```python
from build123d import *

# Parameters (mm, degrees)
BOSS_EXTRUDE1_DEPTH          = 1.5
SKETCH2_W                    = 90
SKETCH2_H                    = 1.5
BOSS_EXTRUDE2_DEPTH          = 36
BOSS_EXTRUDE3_DEPTH          = 1.5
F_6_0_6_DIAMETER_HOLE1_D     = 6
F_6_0_6_DIAMETER_HOLE1_DEPTH = 1.5
F_6_0_6_DIAMETER_HOLE2_D     = 6
F_4_0_4_DIAMETER_HOLE1_D     = 4
F_3_0_3_DIAMETER_HOLE1_D     = 3
FILLET1_R                    = 0.7366
FILLET2_R                    = 2.2366


with BuildPart() as part:
    # Sketch1 → Boss-Extrude1 (new body)
    with BuildSketch(Plane(origin=(-29, 0, 0), x_dir=(0, -1, 0), z_dir=(-1, 0, 0))):
        with BuildLine():
            Line((-9.138054181, -90), (1.5, -90))
            Line((1.5, -90), (1.5, 0))
            Line((1.5, 0), (-2.128893479, 0))
            ThreePointArc((-2.128893479, 0), (-9.130094082, -7.130859089), (-2.128893479, -14.261718178))
            Line((-2.128893479, -14.261718178), (-2.128893479, -41.261718178))
            Line((-2.128893479, -41.261718178), (-3.628893479, -41.261718178))
            ThreePointArc((-3.628893479, -41.261718178), (-5.147993713, -42.802982792), (-5.778257675, -44.873231442))
            ThreePointArc((-5.778257675, -44.873231442), (-5.210002115, -47.08061414), (-3.638283373, -48.73141787))
            Line((-3.638283373, -48.73141787), (-2.138054181, -48.73141787))
            Line((-2.138054181, -48.73141787), (-2.138054181, -75.73141787))
            ThreePointArc((-2.138054181, -75.73141787), (-7.103512649, -77.954400774), (-9.138054181, -83))
            Line((-9.138054181, -83), (-9.138054181, -90))
        make_face()
    extrude(amount=-BOSS_EXTRUDE1_DEPTH)

    # Sketch2 → Boss-Extrude2 (add)
    with BuildSketch(Plane(origin=(-27.5, 0, 0), x_dir=(0, 0, -1), z_dir=(1, 0, 0))):
        with Locations((45, -0.75)):
            Rectangle(SKETCH2_W, SKETCH2_H)
    extrude(amount=BOSS_EXTRUDE2_DEPTH)

    # Sketch3 → Boss-Extrude3 (add)
    with BuildSketch(Plane(origin=(8.5, 0, 0), x_dir=(0, 0, -1), z_dir=(1, 0, 0))):
        with BuildLine():
            Line((0, -1.5), (0, 2.128893479))
            ThreePointArc((0, 2.128893479), (7.130859089, 9.130094082), (14.261718178, 2.128893479))
            Line((14.261718178, 2.128893479), (41.261718178, 2.128893479))
            Line((41.261718178, 2.128893479), (41.261718178, 3.628893479))
            ThreePointArc((41.261718178, 3.628893479), (42.802982792, 5.147993713), (44.873231442, 5.778257675))
            ThreePointArc((44.873231442, 5.778257675), (47.08061414, 5.210002115), (48.73141787, 3.638283373))
            Line((48.73141787, 3.638283373), (48.73141787, 2.138054181))
            Line((48.73141787, 2.138054181), (75.73141787, 2.138054181))
            ThreePointArc((75.73141787, 2.138054181), (77.954400774, 7.103512649), (83, 9.138054181))
            Line((83, 9.138054181), (90, 9.138054181))
            Line((90, 9.138054181), (90, -1.5))
            Line((90, -1.5), (0, -1.5))
        make_face()
    extrude(amount=BOSS_EXTRUDE3_DEPTH)

    # Ø6.0 (6) Diameter Hole1
    with Locations(Plane.ZY.offset(-8.5)):
        with Locations((-6.845764439, 4.481725402), (-83, 4.638054181)):
            Hole(F_6_0_6_DIAMETER_HOLE1_D / 2, depth=F_6_0_6_DIAMETER_HOLE1_DEPTH)

    # Ø6.0 (6) Diameter Hole2 (through all)
    with Locations(Plane(origin=(-27.5, 0, 0), x_dir=(0, 0, -1), z_dir=(1, 0, 0))):
        with Locations((83, 4.638054181), (6.845764439, 4.481725402)):
            Hole(F_6_0_6_DIAMETER_HOLE2_D / 2)

    # Ø4.0 (4) Diameter Hole1 (through all)
    with Locations(Plane(origin=(0, 0, 0), x_dir=(1, 0, 0), z_dir=(0, 1, 0))):
        with Locations((-19.5, 76), (0.5, 76)):
            Hole(F_4_0_4_DIAMETER_HOLE1_D / 2)

    # Ø3.0 (3) Diameter Hole1 (through all)
    with Locations(Plane(origin=(0, 0, 0), x_dir=(1, 0, 0), z_dir=(0, 1, 0))):
        with Locations((-9.5, 6), (-9.5, 23)):
            Hole(F_3_0_3_DIAMETER_HOLE1_D / 2)

    # Fillet1
    fillet1_edges = [part.edges().sort_by_distance(p)[0] for p in [
        (-27.5, 0, -45),
        (8.5, 0, -45),
    ]]
    fillet(fillet1_edges, radius=FILLET1_R)

    # Fillet2
    fillet2_edges = [part.edges().sort_by_distance(p)[0] for p in [
        (-29, -1.5, -45),
        (10, -1.5, -45),
    ]]
    fillet(fillet2_edges, radius=FILLET2_R)


solid = part.part
```
Build history of the part. All positions in model axes, mm. A direction names the side the tool comes from. Round coordinates to 2 decimals unless told otherwise and drop trailing zeros. Order: outer loops, then holes, each group sorted by start corner. A loop starts at its lowest first (then second) coordinate and runs counter-clockwise, first axis right, second up. Notation, with made-up numbers: (-30.75, -40) -> (-22.75, -40) arc R18 ccw to (-22.75, -35) -> close; hole circle Ø1 at (49.5, 58). An arc over 180 degrees is marked (long way). Answer in a Markdown table with one row per item.
1) Wall check: L1, parallel to Z at x = -9.5, y = -0.55; L2, parallel to X at y = 4, z = -42; L3, parallel to Y at x = -6, z = -17. Give the ranges that are in metal, low to high.
Values:
| item | result |
|---|---|
| L1 | -90 to -24.5, -21.5 to -7.5, -4.5 to 0 |
| L2 | -29 to -27.5, 8.5 to 10 |
| L3 | -1.5 to 0 |
2) Band-saw the part on D-D on z = -82. Give the cut face in (x, y).
Values:
| item | result |
|---|---|
| outline | (-29, 0.74) arc R2.24 ccw to (-26.76, -1.5) -> (7.76, -1.5) arc R2.24 ccw to (10, 0.74) -> (10, 1.81) -> (8.5, 1.81) -> (8.5, 0.74) arc R0.74 cw to (7.76, 0) -> (-26.76, 0) arc R0.74 cw to (-27.5, 0.74) -> (-27.5, 1.81) -> (-29, 1.81) -> close; (-29, 7.47) -> (-27.5, 7.47) -> (-27.5, 9.07) -> (-29, 9.07) -> close; (8.5, 7.47) -> (10, 7.47) -> (10, 9.07) -> (8.5, 9.07) -> close |
3) Band-saw the part on C-C on z = -32. Give the cut face in (x, y).
Values:
| item | result |
|---|---|
| outline | (-29, 0.74) arc R2.24 ccw to (-26.76, -1.5) -> (7.76, -1.5) arc R2.24 ccw to (10, 0.74) -> (10, 2.13) -> (8.5, 2.13) -> (8.5, 0.74) arc R0.74 cw to (7.76, 0) -> (-26.76, 0) arc R0.74 cw to (-27.5, 0.74) -> (-27.5, 2.13) -> (-29, 2.13) -> close |
4) Pin check, flat tips, straight feed: P1, Ø5.5, axis at y = 4.64, z = -83, coming from the +X side; P2, Ø1.2, axis at x = 9.5, z = -33, coming from the +Y side; P3, Ø10.5, axis at x = -2.5, z = -42.5, coming from the +Y side. Stop position of each tip, or through.
Values:
| item | result |
|---|---|
| P1 | through |
| P2 | y = 2.13 |
| P3 | y = 0 |
5) Mould opens along Y. For faces 4 (the cylindrical face through (-28.26, 9.13, -6.98)), 5 (the flat face through (9, 3, -41.262)), 6 (the cylindrical face through (9.26, 7.01, -8.46)) say: released by +Y, released by -Y, zero draft, split by the parting line, or undercut.
Values:
| item | result |
|---|---|
| face 4 | released by +Y |
| face 5 | zero draft |
| face 6 | undercut |
6) Band-saw the part on B-B on x = -9.5. Give the cut face in (y, z), and give its area (3 significant figures).
Values:
| item | result |
|---|---|
| outline | (-1.5, -90) -> (0, -90) -> (0, -24.5) -> (-1.5, -24.5) -> close; (-1.5, -21.5) -> (0, -21.5) -> (0, -7.5) -> (-1.5, -7.5) -> close; (-1.5, -4.5) -> (0, -4.5) -> (0, 0) -> (-1.5, 0) -> close |
| area | 126 mm2 |
7) Which spindle directions (+Z, -Z, +X, -X, +Y, -Y) get a long thin tool onto all of the face, cutting with end or side? Do faces 1 (the flat face through (9, 2.138, -62)), 2 (the flat face through (10, 3.4, -48.5)), 3 (the flat face through (-27.5, 3, -48)). Say none if no direction does.
Values:
| item | result |
|---|---|
| face 1 | +X, -X, +Y |
| face 2 | +Z, -Z, +X, +Y, -Y |
| face 3 | +Z, -Z, +Y |
8) Band-saw the part on A-A on x = -19.5. Give the cut face in (y, z).
Values:
| item | result |
|---|---|
| outline | (-1.5, -90) -> (0, -90) -> (0, -78) -> (-1.5, -78) -> close; (-1.5, -74) -> (0, -74) -> (0, 0) -> (-1.5, 0) -> close |
